Here's the drawing with two shaded views (mm, measured from the low corner). I have some questions. Round coordinates to 2 decimals unless told otherwise and drop trailing zeros. Write each loop counter-clockwise with the first axis right and the second up, starting at its lowest first coordinate (ties: lowest second). Pieces come first, ordered by that corner, then holes. Notation, with made-up numbers: (-23.75, 29) -> (2.25, 29) arc R10 cw to (2.25, 44) -> close; hole circle Ø11 at (-12, 69). An arc over 180 degrees is marked (long way). Use CSV: the item, a comma, the result in double quotes.
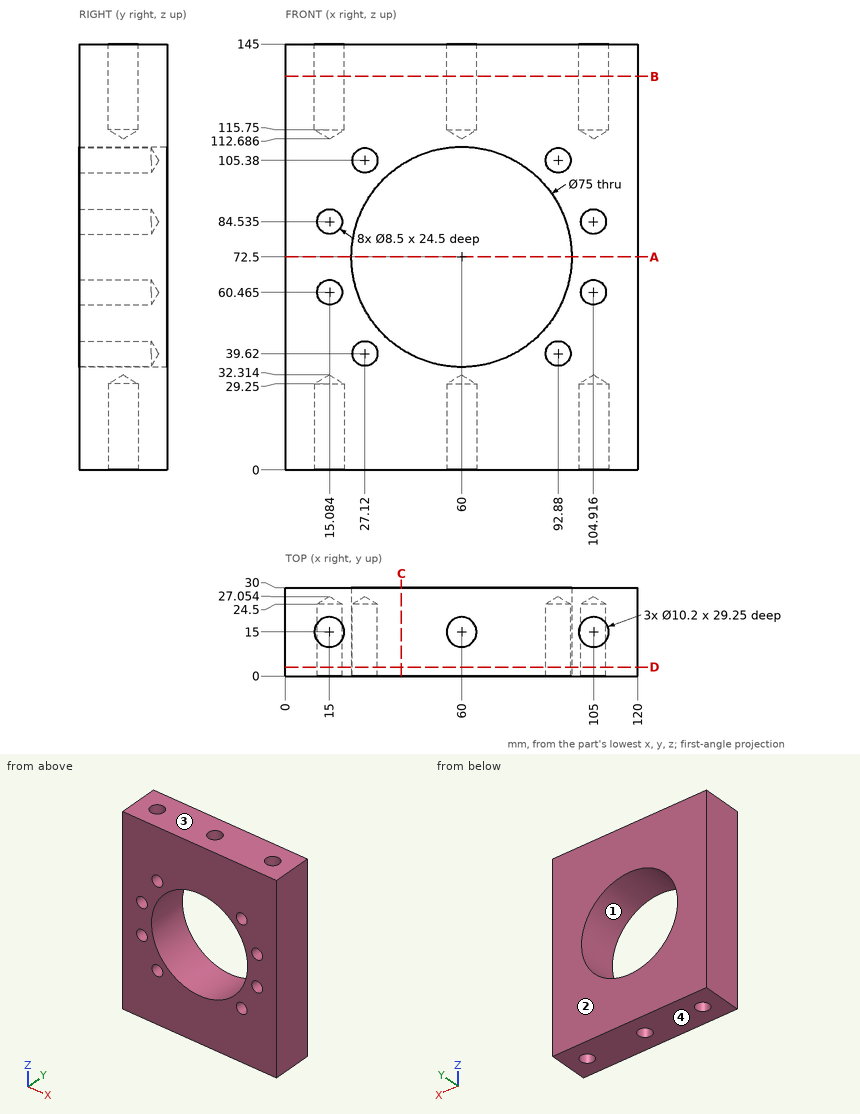
Q1. Suppose I cut it at D-D (y = 3). Count the separate pieces of the cut face and the enclosed holes in it, and give its area (3 significant figures).
Resolved:
separate pieces,"1"
enclosed holes,"9"
area,"12,500 mm^2"
Q2. Please list where these lines run through material, in increasing order: probe 1 along Z at (x, y) = (105, 2) (1 decimal); probe 2 along X at (y, z) = (14.5, 131) (1 decimal); probe 3 along Z at (x, y) = (61.5, 20.25).
Resolved:
probe 1,"z = 0 to 56.2, 64.7 to 80.3, 88.8 to 145"
probe 2,"x = 0 to 9.9, 20.1 to 54.9, 65.1 to 99.9, 110.1 to 120"
probe 3,"z = 0 to 35.03, 109.97 to 145"
Q3. Suppose I cut it at B-B (z = 134). Write out the boundary of the cut face in (x, y).
Resolved:
outline,"(0, 0) -> (120, 0) -> (120, 30) -> (0, 30) -> close; hole circle Ø10.2 at (15, 15); hole circle Ø10.2 at (60, 15); hole circle Ø10.2 at (105, 15)"
Q4. Suppose I cut it at C-C (x = 39.5). Write out the boundary of the cut face in (y, z).
Resolved:
outline,"(0, 0) -> (30, 0) -> (30, 41.1) -> (0, 41.1) -> close; (0, 103.9) -> (30, 103.9) -> (30, 145) -> (0, 145) -> close"
Q5. Will these pins go through, and if not, where does the flat tip stop? P1, Ø11.5, axis at x = 60, y = 15, coming from the -Z side; P2, Ø6, axis at x = 15, y = 15, coming from the +Z side; P3, Ø5, axis at x = 92.88, z = 105.38, coming from the -Y side; P4, Ø7, axis at x = 104.92, z = 60.46, coming from the -Y side.
Resolved:
P1,"stops at z = 0"
P2,"stops at z = 114.49"
P3,"stops at y = 25.55"
P4,"stops at y = 24.95"
Q6. If we mould it in two halves opening along Z, with no side actions, what happens to the marked faces 1, 2, 3 and 4? For each: released by +Z, released by -Z, zero draft, split by the parting line, or undercut.
Resolved:
face 1,"undercut"
face 2,"zero draft"
face 3,"released by +Z"
face 4,"released by -Z"
Q7. Suppose I cut it at A-A (z = 72.5). Write out the boundary of the cut face in (x, y), and give its area (3 significant figures).
Resolved:
outline,"(0, 0) -> (22.5, 0) -> (22.5, 30) -> (0, 30) -> close; (97.5, 0) -> (120, 0) -> (120, 30) -> (97.5, 30) -> close"
area,"1,350 mm^2"
